The listing builds one solid part. Answer for the finished solid, in the listing's coordinates (mm). A direction names the side the tool comes from. Coordinates: 2 decimals unless noted, no trailing zeros. Order: outer loops, then holes, each group sorted by start corner. A loop starts at its lowest first (then second) coordinate and runs counter-clockwise, first axis right, second up. Notation, with made-up numbers: (15, 16.5) -> (63, 16.5) arc R20 cw to (63, 43.5) -> close; hole circle Ø8 at (34.5, 75.25). An arc over 180 degrees is marked (long way). One line per question, with ' | ' between items.
from build123d import *

# Parameters (mm, degrees)
SKETCH_1_R      = 1.55
EXTRUDE_1_DEPTH = 2
FILLET_1_R      = 2


with BuildPart() as part:
    # 草图1 → 凸台-拉伸1 (new body)
    with BuildSketch(Plane(origin=(0, 0, 0), x_dir=(1, 0, 0), z_dir=(0, 1, 0))):
        with BuildLine():
            Line((41.213806874, 33.138893752), (53.711075827, -1.197070502))
            ThreePointArc((53.711075827, -1.197070502), (58.197070502, -3.288924173), (60.288924173, 1.197070502))
            Line((60.288924173, 1.197070502), (46.953457431, 37.835964254))
            ThreePointArc((46.953457431, 37.835964254), (45.672050785, 39.505925907), (43.664533258, 40.138893752))
            Line((43.664533258, 40.138893752), (-43.664533258, 40.138893752))
            ThreePointArc((-43.664533258, 40.138893752), (-45.672050785, 39.505925907), (-46.953457431, 37.835964254))
            Line((-46.953457431, 37.835964254), (-60.288924173, 1.197070502))
            ThreePointArc((-60.288924173, 1.197070502), (-58.197070502, -3.288924173), (-53.711075827, -1.197070502))
            Line((-53.711075827, -1.197070502), (-41.213806874, 33.138893752))
            Line((-41.213806874, 33.138893752), (41.213806874, 33.138893752))
        make_face()
        with Locations(Location((43.664533258, 36.638893752, 0), (0, 0, 270))):
            Circle(SKETCH_1_R, mode=Mode.SUBTRACT)
        with Locations(Location((57, 0, 0), (0, 0, 270))):
            Circle(SKETCH_1_R, mode=Mode.SUBTRACT)
        with Locations(Location((29.110533258, 36.638893752, 0), (0, 0, 270))):
            Circle(SKETCH_1_R, mode=Mode.SUBTRACT)
        with Locations(Location((36.387533258, 36.638893752, 0), (0, 0, 270))):
            Circle(SKETCH_1_R, mode=Mode.SUBTRACT)
        with Locations(Location((-36.387533258, 36.638893752, 0), (0, 0, 270))):
            Circle(SKETCH_1_R, mode=Mode.SUBTRACT)
        with Locations(Location((-29.110533258, 36.638893752, 0), (0, 0, 270))):
            Circle(SKETCH_1_R, mode=Mode.SUBTRACT)
        with Locations(Location((-21.833533258, 36.638893752, 0), (0, 0, 270))):
            Circle(SKETCH_1_R, mode=Mode.SUBTRACT)
        with Locations(Location((-14.556533258, 36.638893752, 0), (0, 0, 270))):
            Circle(SKETCH_1_R, mode=Mode.SUBTRACT)
        with Locations(Location((-7.279533258, 36.638893752, 0), (0, 0, 270))):
            Circle(SKETCH_1_R, mode=Mode.SUBTRACT)
        with Locations(Location((0, 36.638893752, 0), (0, 0, 270))):
            Circle(SKETCH_1_R, mode=Mode.SUBTRACT)
        with Locations(Location((7.279533258, 36.638893752, 0), (0, 0, 270))):
            Circle(SKETCH_1_R, mode=Mode.SUBTRACT)
        with Locations(Location((14.556533258, 36.638893752, 0), (0, 0, 270))):
            Circle(SKETCH_1_R, mode=Mode.SUBTRACT)
        with Locations(Location((21.833533258, 36.638893752, 0), (0, 0, 270))):
            Circle(SKETCH_1_R, mode=Mode.SUBTRACT)
        with Locations(Location((-43.664533258, 36.638893752, 0), (0, 0, 270))):
            Circle(SKETCH_1_R, mode=Mode.SUBTRACT)
        with Locations(Location((-57, 0, 0), (0, 0, 270))):
            Circle(SKETCH_1_R, mode=Mode.SUBTRACT)
    extrude(amount=EXTRUDE_1_DEPTH)

    # 圆角1
    fillet_1_edges = [part.edges().sort_by_distance(p)[0] for p in [
        (-41.213806874, 1, -33.138893752),
        (41.213806874, 1, -33.138893752),
    ]]
    fillet(fillet_1_edges, radius=FILLET_1_R)


solid = part.part
Item 1: Determine the mould class of faces 3 (the face through (-20.527, 0.986, -35.806)), 4 (the face through (-47.786, 0.986, -15.082)), 5 (the face through (53.7, 1, -19.3)) for opening direction Z: pulls with the +Z half, pulls with the -Z half, needs draft (parallel to the pull), parting line crosses it, or undercut.
Computed values:
face 3: undercut | face 4: pulls with the +Z half | face 5: pulls with the -Z half
Item 2: Section D-D, the plane y = 0.8 is taken. Count the separate pieces of the cut face and the enclosed holes in it, plus the area to 3 significant figures.
Computed values:
separate pieces: 1 | enclosed holes: 15 | area: 1,080 mm^2
Item 3: Section A-A, the plane z = 0 is taken. Give the vertices of the cut face in (x, y), plus the area to 3 significant figures.
Computed values:
outline: (-60.5, 0) -> (-58.55, 0) -> (-58.55, 2) -> (-60.5, 2) -> close; (-55.45, 0) -> (-53.28, 0) -> (-53.28, 2) -> (-55.45, 2) -> close; (53.28, 0) -> (55.45, 0) -> (55.45, 2) -> (53.28, 2) -> close; (58.55, 0) -> (60.5, 0) -> (60.5, 2) -> (58.55, 2) -> close | area: 16.5 mm^2
Item 4: Find the intervals of material crossed by L1, parallel to X at y = 1.05, z = 0; L2, parallel to X at y = 0.5, z = -8.5; L3, parallel to X at y = 0.95, z = 1, in increasing order.
Computed values:
L1: x = -60.5 to -58.55, -55.45 to -53.28, 53.28 to 55.45, 58.55 to 60.5 | L2: x = -57.63 to -50.18, 50.18 to 57.63 | L3: x = -60.35 to -58.18, -55.82 to -53.64, 53.64 to 55.82, 58.18 to 60.35
Item 5: Section B-B, the plane x = -57 is taken. Give the vertices of the cut face in (y, z).
Computed values:
outline: (0, -10.23) -> (2, -10.23) -> (2, -1.55) -> (0, -1.55) -> close; (0, 1.55) -> (2, 1.55) -> (2, 3.5) -> (0, 3.5) -> close
Item 6: For faces 1 (the face through (47.62, 0.99, -15.54)), 2 (the face through (-14.09, 0.99, -35.16)), determine the directions among +Z, -Z, +X, -X, +Y, -Y from which every point of the face is accessible in a straight line to the end or side of a thin tool.
Computed values:
face 1: +Z, +Y, -Y | face 2: +Y, -Y
Item 7: Section C-C, the plane z = -28 is taken. Give the vertices of the cut face in (x, y).
Computed values:
outline: (-50.53, 0) -> (-43.08, 0) -> (-43.08, 2) -> (-50.53, 2) -> close; (43.08, 0) -> (50.53, 0) -> (50.53, 2) -> (43.08, 2) -> close
